from build123d import *

# Parameters (mm, degrees)
SKETCH1_W               = 30
SKETCH1_H               = 30
BOSS_EXTRUDE1_DEPTH     = 2
SKETCH2_R               = 6
BOSS_EXTRUDE2_DEPTH     = 8
SKETCH4_R               = 0.5
CUT_EXTRUDE1_DEPTH      = 10
SKETCH6_R               = 2.5
CUT_EXTRUDE3_DEPTH      = 9
CUT_EXTRUDE4_DEPTH      = 0.1
CUT_EXTRUDE4_DEPTH_BACK = 4
SKETCH7_R               = 0.5
SKETCH8_OUTSIDE_W       = 40.718
SKETCH8_OUTSIDE_H       = 40.718
SKETCH8_OUTSIDE_W_2     = 15.543966854
SKETCH8_OUTSIDE_H_2     = 10
CUT_EXTRUDE5_DEPTH      = 8
M3_TAPPED_HOLE1_D       = 2.5
M3_TAPPED_HOLE1_DEPTH   = 3
M3_TAPPED_HOLE1_TIP     = 0.751075774
M2_5_TAPPED_HOLE1_D     = 2.05


with BuildPart() as part:
    # Sketch1 → Boss-Extrude1 (new body)
    with BuildSketch(Plane.XY):
        Rectangle(SKETCH1_W, SKETCH1_H)
    extrude(amount=BOSS_EXTRUDE1_DEPTH)

    # Sketch2 → Boss-Extrude2 (add)
    with BuildSketch(Plane(origin=(0, 0, 0), x_dir=(-1, 0, 0), z_dir=(0, 0, -1))):
        Circle(SKETCH2_R)
    extrude(amount=BOSS_EXTRUDE2_DEPTH)

    # Sketch4 → Cut-Extrude1 (cut)
    with BuildSketch(Plane.XY.offset(2)):
        with Locations((-12, 12)):
            Circle(SKETCH4_R)
        with Locations((12, 12)):
            Circle(SKETCH4_R)
        with Locations((12, -12)):
            Circle(SKETCH4_R)
        with Locations((-12, -12)):
            Circle(SKETCH4_R)
    extrude(amount=-CUT_EXTRUDE1_DEPTH, mode=Mode.SUBTRACT)

    # Sketch6 → Cut-Extrude3 (cut)
    with BuildSketch(Plane(origin=(0, 0, -8), x_dir=(-1, 0, 0), z_dir=(0, 0, -1))):
        Circle(SKETCH6_R)
    extrude(amount=-CUT_EXTRUDE3_DEPTH, mode=Mode.SUBTRACT)

    # Sketch7 → Cut-Extrude4 (cut, two sides: drawn at the far end of the back side and taken through both)
    with BuildSketch(Plane(origin=(0, 0, 0), x_dir=(1, 0, 0), z_dir=(0, 1, 0)).offset(-CUT_EXTRUDE4_DEPTH_BACK)):
        with Locations(Location((0, 5.5, 0), (0, 0, 270))):
            Circle(SKETCH7_R)
    extrude(amount=CUT_EXTRUDE4_DEPTH + CUT_EXTRUDE4_DEPTH_BACK, mode=Mode.SUBTRACT)

    # Sketch8 outside → Cut-Extrude5 (cut)
    with BuildSketch(Plane(origin=(0, 0, -8), x_dir=(-1, 0, 0), z_dir=(0, 0, -1))):
        Rectangle(SKETCH8_OUTSIDE_W, SKETCH8_OUTSIDE_H)
        Rectangle(SKETCH8_OUTSIDE_W_2, SKETCH8_OUTSIDE_H_2, mode=Mode.SUBTRACT)
    extrude(amount=-CUT_EXTRUDE5_DEPTH, mode=Mode.SUBTRACT)

    # M3 Tapped Hole1
    with Locations(Plane(origin=(0, -5, 0), x_dir=(-1, 0, 0), z_dir=(0, -1, 0))):
        with Locations((0, 5.5)):
            Hole(M3_TAPPED_HOLE1_D / 2, depth=M3_TAPPED_HOLE1_DEPTH)
            with Locations((0, 0, -(M3_TAPPED_HOLE1_DEPTH + M3_TAPPED_HOLE1_TIP / 2))):  # 118° drill point
                Cone(0, M3_TAPPED_HOLE1_D / 2, M3_TAPPED_HOLE1_TIP, mode=Mode.SUBTRACT)

    # M2.5 Tapped Hole1 (through all)
    with Locations(Plane.XY.offset(2)):
        with Locations((12, 12), (12, -12), (-12, -12), (-12, 12)):
            Hole(M2_5_TAPPED_HOLE1_D / 2)


solid = part.part
Here's how the part is built. I have some questions about the finished solid (model axes, mm). A direction names the side the tool comes from. Coordinates: 2 decimals unless noted, no trailing zeros. Order: outer loops, then holes, each group sorted by start corner. A loop starts at its lowest first (then second) coordinate and runs counter-clockwise, first axis right, second up. Notation, with made-up numbers: (-3, 59) -> (48, 59) arc R24 cw to (48, 84) -> close; hole circle Ø8 at (-21, 85.25). An arc over 180 degrees is marked (long way). Answer in a Markdown table with one row per item.
(1) I want a section at A-A on x = -12. List the corners of the cut face in (y, z) for me (3 decimals), then the cut area to 3 significant figures.
Answer key:
| item | result |
|---|---|
| outline | (-15, 0) -> (-13.025, 0) -> (-13.025, 2) -> (-15, 2) -> close; (-10.975, 0) -> (10.975, 0) -> (10.975, 2) -> (-10.975, 2) -> close; (13.025, 0) -> (15, 0) -> (15, 2) -> (13.025, 2) -> close |
| area | 51.8 mm^2 |
(2) Will these pins go through, and if not, where does the flat tip stop? pin 1 Ø2.5 at (x, y) = (12, -12) entering from -Z; pin 2 Ø2 at (x, z) = (-2.5, -3) entering from -Y; pin 3 Ø3 at (x, y) = (0, 0) entering from -Z.
Answer key:
| item | result |
|---|---|
| pin 1 | z = 0 |
| pin 2 | y = -5 |
| pin 3 | z = 1 |
(3) I want a section at D-D on z = -1.5. List the corners of the cut face in (x, y) for me, then the cut area to 3 significant figures.
Answer key:
| item | result |
|---|---|
| outline | (-3.32, -5) -> (3.32, -5) arc R6 ccw to (3.32, 5) -> (-3.32, 5) arc R6 ccw to start; hole circle Ø5 at (0, 0) |
| area | 84.5 mm^2 |
(4) Thinking about a two-plate mould opening in Y: for faces 6 (the face through (0, 5, -4)), 7 (the face through (-0.27, -3.56, -4.28)), 8 (the face through (0.33, 2.48, -3.56)), which applies, +Y half, -Y half, draft (parallel to the pull), parting line (faces both ways), or undercut?
Answer key:
| item | result |
|---|---|
| face 6 | +Y half |
| face 7 | draft |
| face 8 | undercut |
(5) I want a section at C-C on y = 0. List the corners of the cut face in (x, z) for me.
Answer key:
| item | result |
|---|---|
| outline | (-15, 0) -> (-6, 0) -> (-6, -8) -> (-2.5, -8) -> (-2.5, 1) -> (2.5, 1) -> (2.5, -8) -> (6, -8) -> (6, 0) -> (15, 0) -> (15, 2) -> (-15, 2) -> close |
(6) Please list where these lines run through material, in increasing order: probe 1 along Y at (x, z) = (-12, 0.6) (3 decimals); probe 2 along Z at (x, y) = (-12.5, 10); probe 3 along Y at (x, z) = (-1, -3).
Answer key:
| item | result |
|---|---|
| probe 1 | -15 to -13.025, -10.975 to 10.975, 13.025 to 15 |
| probe 2 | 0 to 2 |
| probe 3 | -5 to -2.29, 2.29 to 5 |
(7) On a 3-axis mill with a long thin cutter (end or side, diameter ignored), from which of +Z, -Z, +X, -X, +Y, -Y can I reach the whole of each face in a straight line? I mean faces 1 (the face through (6, 0, -4)), 2 (the face through (0, 0, 1)), 3 (the face through (0, -5, -4)), 4 (the face through (-3, 0, -8)), 5 (the face through (-6, 0, -4)). Say none if no direction works.
Answer key:
| item | result |
|---|---|
| face 1 | -Z, +X |
| face 2 | -Z |
| face 3 | -Z, +X, -X, -Y |
| face 4 | -Z, +X, -X, +Y, -Y |
| face 5 | -Z, -X |
